The model under review builds one solid part; all positions refer to its coordinate system, in mm. A direction names the side the tool comes from. Round coordinates to 2 decimals unless told otherwise and drop trailing zeros. Write each loop counter-clockwise with the first axis right and the second up, starting at its lowest first coordinate (ties: lowest second). Pieces come first, ordered by that corner, then holes.
Item 1: To check wall thickness, follow L1, parallel to Y at x = 3.35, z = 6; L2, parallel to Y at x = 7.7, z = 6; L3, parallel to X at y = -23.5, z = -8.25. State the ranges of each line that lie inside material, in increasing order.
Item 2: Add section B-B (z = 6). Give the boundary of the cut face in (x, y), plus the area to 3 significant figures.
Item 3: Machinability: for faces 1 (the face through (1, -18, 0)), 2 (the face through (5.4, 18, -8)), 3 (the face through (2.662, 18.004, 7.038)), which of the approach directions +Z, -Z, +X, -X, +Y, -Y give a long, thin tool a straight path to every point of the face, cutting with its end or side? Answer none if there is none.
Item 4: Add section C-C (y = -24). Give the boundary of the cut face in (x, z).
Item 5: Draft analysis for pull direction Z (two halves, no side actions). For faces 4 (the face through (4.9, 29, -11.5)), 5 (the face through (5, 0, 12.5)), 6 (the face through (2, -24, 0)), 7 (the face through (7.732, 23.966, -5.479)), state which applies: +Z half, -Z half, draft (parallel to the pull), parting line (faces both ways), or undercut.
Item 6: Add section A-A (x = 4.25). Give the boundary of the cut face in (y, z), plus the area to 3 significant figures.
Item 7: Clearance check with flat-ended pins moving along their axes: pin 1 Ø7 at (y, z) = (20, 6) entering from +X; pin 2 Ø1 at (x, z) = (1, -4) entering from -Y; pin 3 Ø6 at (y, z) = (-26, 3.5) entering from -X. State where each tip first meets the part, or that it passes through.
Item 8: Add section D-D (y = 20). Give the boundary of the cut face in (x, z).
```python
from build123d import *

# Parameters (mm, degrees)
SKETCH1_W                                            = 25
SKETCH1_H                                            = 60
BOSS_EXTRUDE1_DEPTH                                  = 10
SKETCH4_W                                            = 25
SKETCH4_H                                            = 12
CUT_EXTRUDE3_DEPTH                                   = 2
CBORE_FOR_M4_HEXAGON_SOCKET_HEAD_CAP_SCR_D           = 4.5
CBORE_FOR_M4_HEXAGON_SOCKET_HEAD_CAP_SCR_CBORE_D     = 8
CBORE_FOR_M4_HEXAGON_SOCKET_HEAD_CAP_SCR_CBORE_DEPTH = 4.6
CBORE_FOR_M4_HEXAGON_SOCKET_HEAD_CAP_2_D             = 4.5
CBORE_FOR_M4_HEXAGON_SOCKET_HEAD_CAP_2_CBORE_D       = 8
CBORE_FOR_M4_HEXAGON_SOCKET_HEAD_CAP_2_CBORE_DEPTH   = 4.6
CHAMFER1_SIZE                                        = 2


with BuildPart() as part:
    # Sketch1 → Boss-Extrude1 (new body)
    with BuildSketch(Plane(origin=(0, 0, 0), x_dir=(0, 0, -1), z_dir=(1, 0, 0))):
        Rectangle(SKETCH1_W, SKETCH1_H)
    extrude(amount=BOSS_EXTRUDE1_DEPTH)

    # Sketch4 → Cut-Extrude3 (cut)
    with BuildSketch(Plane.ZY):
        with Locations((0, -24)):
            Rectangle(SKETCH4_W, SKETCH4_H)
    extrude(amount=-CUT_EXTRUDE3_DEPTH, mode=Mode.SUBTRACT)

    # CBORE for M4 Hexagon socket head cap scr (through all)
    with Locations(Plane(origin=(10, 0, 0), x_dir=(0, 0, -1), z_dir=(1, 0, 0))):
        with Locations((-6, -24), (6, -24)):
            CounterBoreHole(CBORE_FOR_M4_HEXAGON_SOCKET_HEAD_CAP_SCR_D / 2, CBORE_FOR_M4_HEXAGON_SOCKET_HEAD_CAP_SCR_CBORE_D / 2, CBORE_FOR_M4_HEXAGON_SOCKET_HEAD_CAP_SCR_CBORE_DEPTH)

    # CBORE for M4 Hexagon socket head cap 2 (through all)
    with Locations(Plane(origin=(10, 0, 0), x_dir=(0, 0, -1), z_dir=(1, 0, 0))):
        with Locations((6, 20), (-6, 20)):
            CounterBoreHole(CBORE_FOR_M4_HEXAGON_SOCKET_HEAD_CAP_2_D / 2, CBORE_FOR_M4_HEXAGON_SOCKET_HEAD_CAP_2_CBORE_D / 2, CBORE_FOR_M4_HEXAGON_SOCKET_HEAD_CAP_2_CBORE_DEPTH)

    # Chamfer1
    chamfer1_edges = [part.edges().sort_by_distance(p)[0] for p in [
        (6, -30, -12.5),
        (6, -30, 12.5),
        (5, 30, 12.5),
        (5, 30, -12.5),
    ]]
    chamfer(chamfer1_edges, length=CHAMFER1_SIZE)


solid = part.part
```
Numbers:
1. L1: y = -30 to -26.25, -21.75 to 17.75, 22.25 to 30
1. L2: y = -30 to -28, -20 to 16, 24 to 30
1. L3: x = 2 to 5.4
2. outline: (0, -18) - (2, -18) - (2, -21.75) - (5.4, -21.75) - (5.4, -20) - (10, -20) - (10, 16) - (5.4, 16) - (5.4, 17.75) - (0, 17.75) - close; (0, 22.25) - (5.4, 22.25) - (5.4, 24) - (10, 24) - (10, 30) - (0, 30) - close; (2, -30) - (10, -30) - (10, -28) - (5.4, -28) - (5.4, -26.25) - (2, -26.25) - close
2. area: 463 mm2
3. face 1: +Z, -Z, -X, -Y
3. face 2: +X
3. face 3: +X, -X
4. outline: (2, -12.5) - (10, -12.5) - (10, -10) - (5.4, -10) - (5.4, -8.25) - (2, -8.25) - close; (2, -3.75) - (5.4, -3.75) - (5.4, -2) - (10, -2) - (10, 2) - (5.4, 2) - (5.4, 3.75) - (2, 3.75) - close; (2, 8.25) - (5.4, 8.25) - (5.4, 10) - (10, 10) - (10, 12.5) - (2, 12.5) - close
5. face 4: -Z half
5. face 5: +Z half
5. face 6: draft
5. face 7: undercut
6. outline: (-30, -10.5) - (-28, -12.5) - (28, -12.5) - (30, -10.5) - (30, 10.5) - (28, 12.5) - (-28, 12.5) - (-30, 10.5) - close; hole circle Ø4.5 at (-24, -6); hole circle Ø4.5 at (-24, 6); hole circle Ø4.5 at (20, -6); hole circle Ø4.5 at (20, 6)
6. area: 1,430 mm2
7. pin 1: stops at x = 5.4
7. pin 2: stops at y = -18
7. pin 3: stops at x = 2
8. outline: (0, -12.5) - (10, -12.5) - (10, -10) - (5.4, -10) - (5.4, -8.25) - (0, -8.25) - close; (0, -3.75) - (5.4, -3.75) - (5.4, -2) - (10, -2) - (10, 2) - (5.4, 2) - (5.4, 3.75) - (0, 3.75) - close; (0, 8.25) - (5.4, 8.25) - (5.4, 10) - (10, 10) - (10, 12.5) - (0, 12.5) - close
